The figure shows three views and two pictorial views of one solid part (mm, origin at its lowest corner). Answer the questions. A direction names the side the tool comes from. Round coordinates to 2 decimals unless told otherwise and drop trailing zeros. Order: outer loops, then holes, each group sorted by start corner. A loop starts at its lowest first (then second) coordinate and runs counter-clockwise, first axis right, second up. Notation, with made-up numbers: (30.25, 15) - (87.25, 15) arc R28 cw to (87.25, 34) - close; hole circle Ø11 at (66, 19.25). An arc over 180 degrees is marked (long way). Answer as a JSON object with one key per item and string values. Group by question number.
Q1. A cutting plane is placed at A-A on x = 10. Determine the outline of the cut face in (y, z).
Q2. Consider line 1 (Y direction, x = 10, z = 8.6); line 2 (Y direction, x = 10, z = 4.5); line 3 (X direction, y = 16.5, z = 1.5). Determine where each line is inside the solid, lowest interval first.
Q3. A cutting plane is placed at D-D on z = 1.5. Determine the outline of the cut face in (x, y).
Q4. A tool of negligible diameter and unlimited length cuts with its end or side. For the marked faces 1, 2, 3 and 4, from which of +Z, -Z, +X, -X, +Y, -Y can it reach the whole face along a straight path? Write none if from no direction.
Q5. A cutting plane is placed at C-C on y = 7.5. Determine the outline of the cut face in (x, z), and give its area (3 significant figures).
Q6. Given pin 1 Ø2 at (x, y) = (2.5, 28.5) entering from -Z; pin 2 Ø5.5 at (y, z) = (27.5, 3) entering from +X; pin 3 Ø1.8 at (x, y) = (9.5, 7) entering from +Z; pin 4 Ø1.5 at (y, z) = (28, 2.5) entering from -X, each flat-ended and moving along its own axis, determine where each tip first touches the part or whether it passes through.
Q7. A cutting plane is placed at B-B on z = 7.75. Determine the outline of the cut face in (x, y).
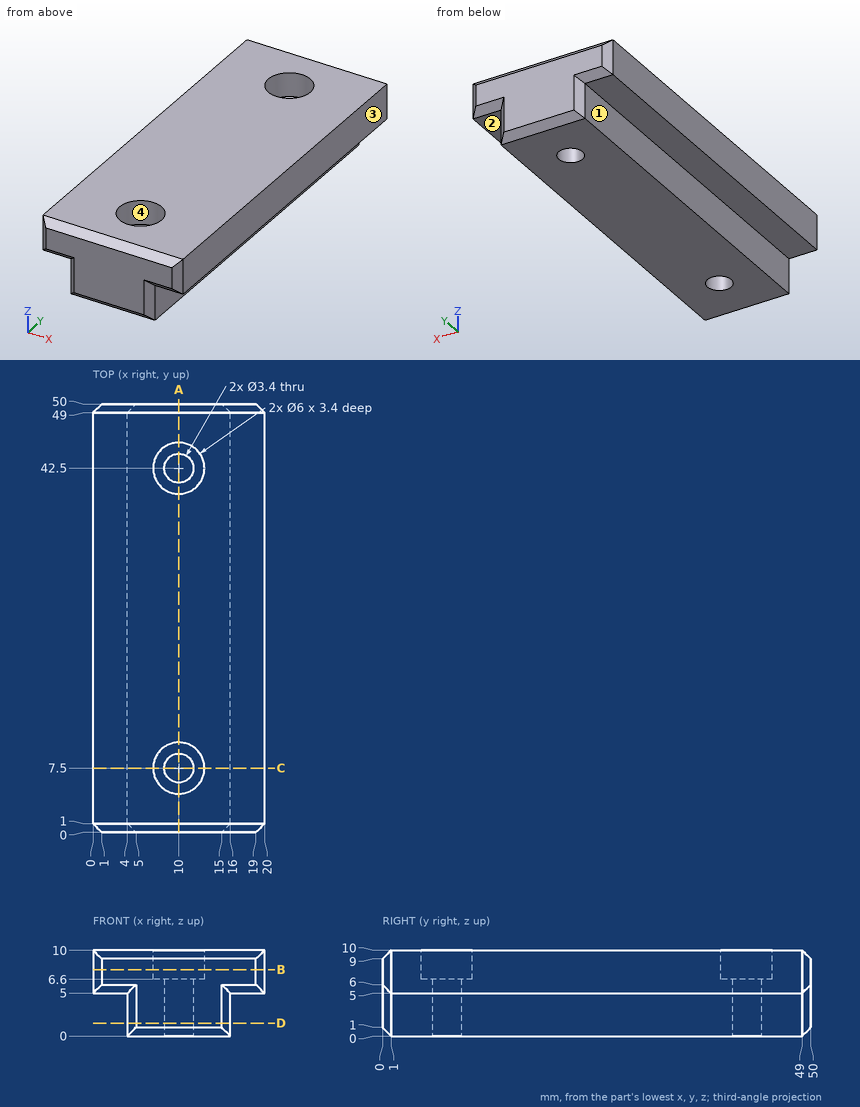
Result set:
{
 "1": {"outline": "(0, 1) - (1, 0) - (5.8, 0) - (5.8, 6.6) - (4.5, 6.6) - (4.5, 10) - (1, 10) - (0, 9) - close; (9.2, 0) - (40.8, 0) - (40.8, 6.6) - (39.5, 6.6) - (39.5, 10) - (10.5, 10) - (10.5, 6.6) - (9.2, 6.6) - close; (44.2, 0) - (49, 0) - (50, 1) - (50, 9) - (49, 10) - (45.5, 10) - (45.5, 6.6) - (44.2, 6.6) - close"},
 "2": {"line 1": "y = 0 to 4.5, 10.5 to 39.5, 45.5 to 50", "line 2": "y = 0 to 5.8, 9.2 to 40.8, 44.2 to 50", "line 3": "x = 4 to 16"},
 "3": {"outline": "(4, 1) - (5, 0) - (15, 0) - (16, 1) - (16, 49) - (15, 50) - (5, 50) - (4, 49) - close; hole circle Ø3.4 at (10, 7.5); hole circle Ø3.4 at (10, 42.5)"},
 "4": {"face 1": "-Z, -X, +Y, -Y", "face 2": "-Z, +X, +Y, -Y", "face 3": "+Z, -Z, +X, +Y, -Y", "face 4": "+Z"},
 "5": {"outline": "(0, 5) - (4, 5) - (4, 0) - (8.3, 0) - (8.3, 6.6) - (7, 6.6) - (7, 10) - (0, 10) - close; (11.7, 0) - (16, 0) - (16, 5) - (20, 5) - (20, 10) - (13, 10) - (13, 6.6) - (11.7, 6.6) - close", "area": "117 mm²"},
 "6": {"pin 1": "stops at z = 5", "pin 2": "stops at x = 20", "pin 3": "passes through", "pin 4": "stops at x = 4"},
 "7": {"outline": "(0, 1) - (1, 0) - (19, 0) - (20, 1) - (20, 49) - (19, 50) - (1, 50) - (0, 49) - close; hole circle Ø6 at (10, 7.5); hole circle Ø6 at (10, 42.5)"}
}
